Verification items for this drawing (mm, ordinates from the low corner). A direction names the side the tool comes from. Round coordinates to 2 decimals unless told otherwise and drop trailing zeros. Write each loop counter-clockwise with the first axis right and the second up, starting at its lowest first coordinate (ties: lowest second). Pieces come first, ordered by that corner, then holes. Notation, with made-up numbers: (-23, -2.5) -> (-18, -2.5) arc R17 cw to (-18, 23.5) -> close; hole circle Ø9 at (-26.5, 58.25). An arc over 180 degrees is marked (long way). Put each result on its own line as item: value. Start each with the question number.
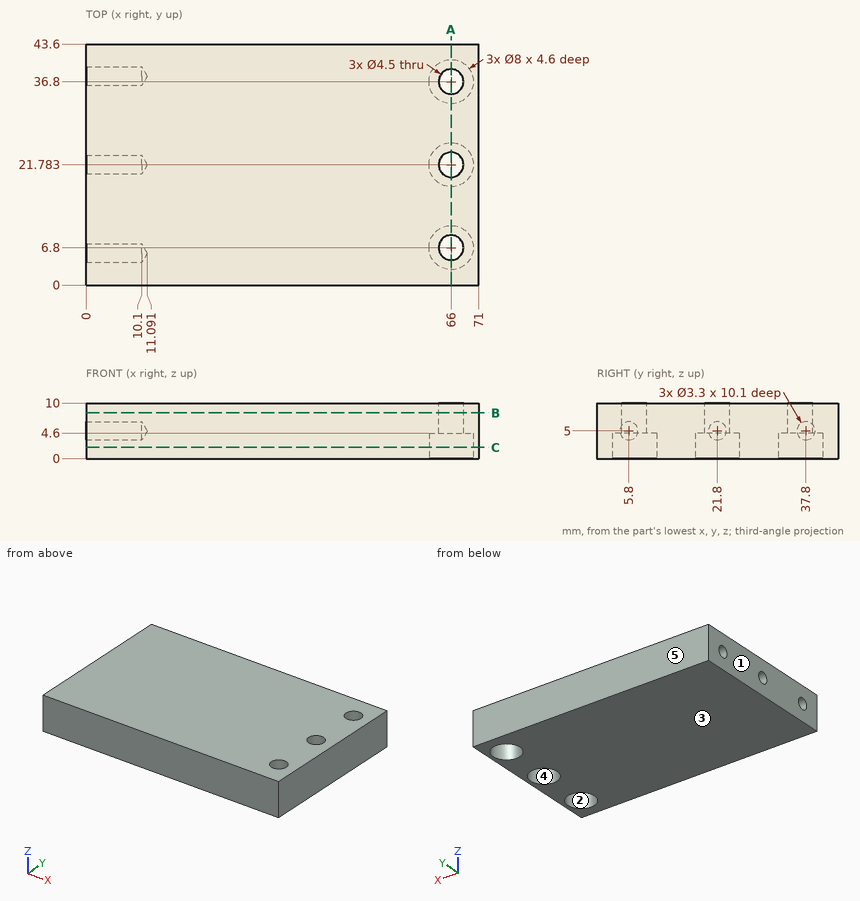
1. Draft check along X on the marked faces 1, 2 and 3. Enter one of: released by +X, released by -X, zero draft, split by the parting line, or undercut.
2. Section check B-B, the plane z = 8.25. Enter the section's corners in (x, y).
3. Gauge pin test, flat ends, axial feed: P1, Ø6.5, axis at x = 66, y = 36.8, coming from the +Z side; P2, Ø6, axis at x = 66, y = 6.8, coming from the -Z side. Record the tip position at first contact, or that the pin passes through.
4. Material ranges on L1, parallel to Y at x = 2.5, z = 5; L2, parallel to Y at x = 66, z = 7; L3, parallel to X at y = 35.5, z = 9.75 (1 decimal), recorded low to high. Write a range as [from, to].
5. Section check A-A, the plane x = 66. Enter the section's corners in (y, z), then the cut area to 3 significant figures.
6. Section check C-C, the plane z = 2. Enter the section's corners in (x, y), then the cut area to 4 significant figures.
7. Access from +Z, -Z, +X, -X, +Y, -Y to the whole of each face (thin tool, end or side, straight path). Record for the marked faces 4 and 5.
Reply:
1. face 1: released by -X
1. face 2: undercut
1. face 3: zero draft
2. outline: (0, 0) -> (71, 0) -> (71, 43.6) -> (0, 43.6) -> close; hole circle Ø4.5 at (66, 6.8); hole circle Ø4.5 at (66, 21.78); hole circle Ø4.5 at (66, 36.8)
3. P1: stops at z = 10
3. P2: stops at z = 4.6
4. L1: y = [0, 4.15], [7.45, 20.15], [23.45, 36.15], [39.45, 43.6]
4. L2: y = [0, 4.55], [9.05, 19.53], [24.03, 34.55], [39.05, 43.6]
4. L3: x = [0, 64.2], [67.8, 71]
5. outline: (0, 0) -> (2.8, 0) -> (2.8, 4.6) -> (4.55, 4.6) -> (4.55, 10) -> (0, 10) -> close; (9.05, 4.6) -> (10.8, 4.6) -> (10.8, 0) -> (17.78, 0) -> (17.78, 4.6) -> (19.53, 4.6) -> (19.53, 10) -> (9.05, 10) -> close; (24.03, 4.6) -> (25.78, 4.6) -> (25.78, 0) -> (32.8, 0) -> (32.8, 4.6) -> (34.55, 4.6) -> (34.55, 10) -> (24.03, 10) -> close; (39.05, 4.6) -> (40.8, 4.6) -> (40.8, 0) -> (43.6, 0) -> (43.6, 10) -> (39.05, 10) -> close
5. area: 253 mm2
6. outline: (0, 0) -> (71, 0) -> (71, 43.6) -> (0, 43.6) -> close; hole circle Ø8 at (66, 6.8); hole circle Ø8 at (66, 21.78); hole circle Ø8 at (66, 36.8)
6. area: 2,945 mm2
7. face 4: -Z
7. face 5: +Z, -Z, +X, -X, +Y
